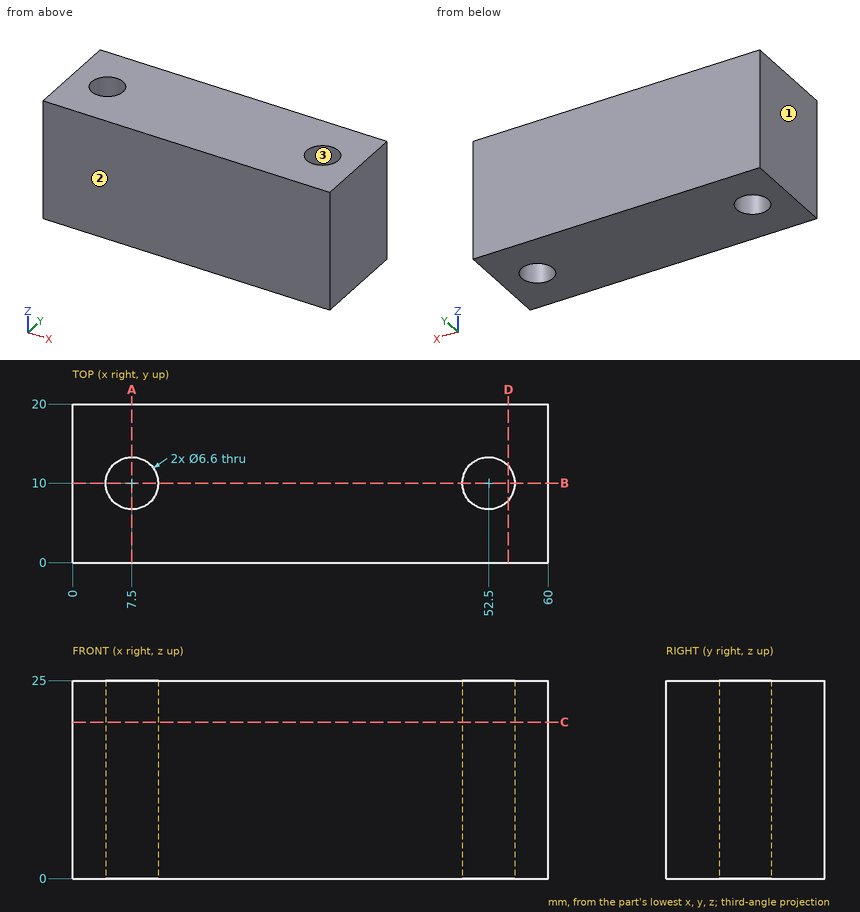
Geometry check sheet. Reference: drawing and pictorial views, mm from the part's lowest x, y, z. Give positions to 0.01 mm unless a question says otherwise; leave off trailing zeros. Loops run counter-clockwise (first coordinate to the right, second up) from the corner with the lowest first, then second, coordinate; pieces in that order, holes last. Notation, with made-up numbers: (72, 34.25) - (101, 34.25) arc R15 cw to (101, 58.25) - close; hole circle Ø2 at (41, 56.5). An arc over 180 degrees is marked (long way). Use CSV: the item, a comma, the result in double quotes. Start each with the question number.
Q1. Section check D-D, the plane x = 55. Record the cut outline in (y, z), and give its area (3 significant figures).
Q2. Section check C-C, the plane z = 19.75. Record the cut outline in (x, y).
Q3. Section check B-B, the plane y = 10. Record the cut outline in (x, z), and give its area (3 significant figures).
Q4. Go/stop test with flat-tipped pins: pin 1 Ø5.5 at (x, y) = (52.5, 10) entering from -Z; pin 2 Ø2 at (y, z) = (10.5, 11) entering from -X. Record where each tip stops, or that it passes through.
Q5. Release check for a two-part mould opening along X. For the marked faces 1, 2 and 3 record: +X half, -X half, draft (parallel to the pull), parting line (faces both ways), or undercut.
Q6. Scan lines: probe 1 along X at (y, z) = (10.25, 15.25); probe 2 along Y at (x, z) = (7.5, 17.25); probe 3 along Y at (x, z) = (51.5, 24). Record each from-to range of solid material in increasing order. Write a range as from..to.
Q7. Section check A-A, the plane x = 7.5. Record the cut outline in (y, z).
Findings below:
1,outline,"(0, 0) - (7.85, 0) - (7.85, 25) - (0, 25) - close; (12.15, 0) - (20, 0) - (20, 25) - (12.15, 25) - close"
1,area,"392 mm^2"
2,outline,"(0, 0) - (60, 0) - (60, 20) - (0, 20) - close; hole circle Ø6.6 at (7.5, 10); hole circle Ø6.6 at (52.5, 10)"
3,outline,"(0, 0) - (4.2, 0) - (4.2, 25) - (0, 25) - close; (10.8, 0) - (49.2, 0) - (49.2, 25) - (10.8, 25) - close; (55.8, 0) - (60, 0) - (60, 25) - (55.8, 25) - close"
3,area,"1,170 mm^2"
4,pin 1,"passes through"
4,pin 2,"stops at x = 0"
5,face 1,"-X half"
5,face 2,"draft"
5,face 3,"undercut"
6,probe 1,"x = 0..4.21, 10.79..49.21, 55.79..60"
6,probe 2,"y = 0..6.7, 13.3..20"
6,probe 3,"y = 0..6.86, 13.14..20"
7,outline,"(0, 0) - (6.7, 0) - (6.7, 25) - (0, 25) - close; (13.3, 0) - (20, 0) - (20, 25) - (13.3, 25) - close"
